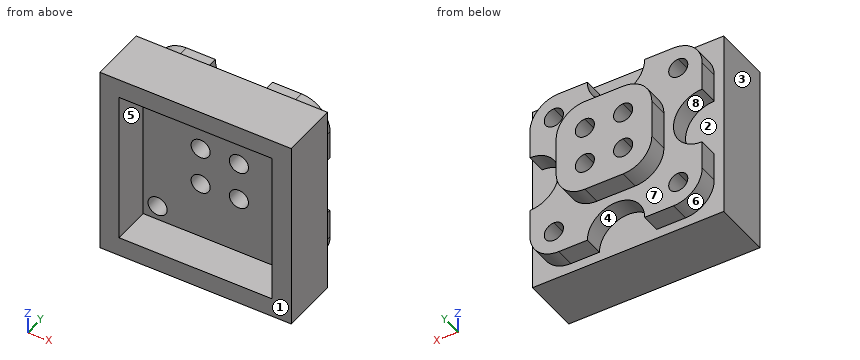
```python
from build123d import *

# Parameters (mm, degrees)
BASE_SQUARE_SKETCH_W        = 100
BASE_SQUARE_SKETCH_H        = 100
BASE_BLOCK_100X100X30_DEPTH = 30
BASE_SHELL_10MM_T           = -10
CROSS_PLATE_SKETCH_R        = 5
CROSS_PLATE_10MM_DEPTH      = 10
PLATE_HOLES_SKETCH_R        = 5
PLATE_ARM_HOLES_4X_DEPTH    = 82.240384046
CENTRE_BOSS_SKETCH_R        = 5
CENTRE_BOSS_10MM_DEPTH      = 10
CENTRE_HOLES_SKETCH_R       = 5
CENTRE_BOSS_HOLES_4X_DEPTH  = 87.602540378


with BuildPart() as part:
    # Base Square Sketch → Base Block 100x100x30 (new body)
    with BuildSketch(Plane(origin=(0, 0, 0), x_dir=(1, 0, 0), z_dir=(0, 1, 0))):
        Rectangle(BASE_SQUARE_SKETCH_W, BASE_SQUARE_SKETCH_H)
    extrude(amount=BASE_BLOCK_100X100X30_DEPTH)

    # Base Shell 10mm
    base_shell_10mm_openings = [part.faces().sort_by_distance(p)[0] for p in [
        (0, 0, 0),
    ]]
    offset(amount=BASE_SHELL_10MM_T, openings=base_shell_10mm_openings, kind=Kind.INTERSECTION)

    # Cross Plate Sketch → Cross Plate 10mm (add)
    with BuildSketch(Plane(origin=(0, 30, 0), x_dir=(1, 0, 0), z_dir=(0, 1, 0))):
        with BuildLine():
            Line((15, 45), (30, 45))
            ThreePointArc((30, 45), (40.606601718, 40.606601718), (45, 30))
            Line((45, 30), (45, 15))
            ThreePointArc((45, 15), (30, 0), (45, -15))
            Line((45, -15), (45, -30))
            ThreePointArc((45, -30), (40.606601718, -40.606601718), (30, -45))
            Line((30, -45), (15, -45))
            ThreePointArc((15, -45), (0, -30), (-15, -45))
            Line((-15, -45), (-30, -45))
            ThreePointArc((-30, -45), (-40.606601718, -40.606601718), (-45, -30))
            Line((-45, -30), (-45, -15))
            ThreePointArc((-45, -15), (-30, 0), (-45, 15))
            Line((-45, 15), (-45, 30))
            ThreePointArc((-45, 30), (-40.606601718, 40.606601718), (-30, 45))
            Line((-30, 45), (-15, 45))
            ThreePointArc((-15, 45), (0, 30), (15, 45))
        make_face()
        with Locations(Location((-32.5, 32.5, 0), (0, 0, 270))):
            Circle(CROSS_PLATE_SKETCH_R, mode=Mode.SUBTRACT)
        with Locations(Location((32.5, 32.5, 0), (0, 0, 270))):
            Circle(CROSS_PLATE_SKETCH_R, mode=Mode.SUBTRACT)
        with Locations(Location((-32.5, -32.5, 0), (0, 0, 270))):
            Circle(CROSS_PLATE_SKETCH_R, mode=Mode.SUBTRACT)
        with Locations(Location((32.5, -32.5, 0), (0, 0, 270))):
            Circle(CROSS_PLATE_SKETCH_R, mode=Mode.SUBTRACT)
    extrude(amount=CROSS_PLATE_10MM_DEPTH)

    # Plate Holes Sketch → Plate Arm Holes 4x (cut, through all)
    with BuildSketch(Plane(origin=(0, 40, 0), x_dir=(1, 0, 0), z_dir=(0, 1, 0))):
        with Locations(Location((-32.5, 32.5, 0), (0, 0, 90))):
            Circle(PLATE_HOLES_SKETCH_R)
        with Locations(Location((32.5, 32.5, 0), (0, 0, 90))):
            Circle(PLATE_HOLES_SKETCH_R)
        with Locations(Location((32.5, -32.5, 0), (0, 0, 90))):
            Circle(PLATE_HOLES_SKETCH_R)
        with Locations(Location((-32.5, -32.5, 0), (0, 0, 90))):
            Circle(PLATE_HOLES_SKETCH_R)
    extrude(amount=-PLATE_ARM_HOLES_4X_DEPTH, mode=Mode.SUBTRACT)

    # Centre Boss Sketch → Centre Boss 10mm (add)
    with BuildSketch(Plane(origin=(0, 40, 0), x_dir=(1, 0, 0), z_dir=(0, 1, 0))):
        with BuildLine():
            Line((-25, 10), (-25, -10))
            ThreePointArc((-25, -10), (-20.606601718, -20.606601718), (-10, -25))
            Line((-10, -25), (10, -25))
            ThreePointArc((10, -25), (20.606601718, -20.606601718), (25, -10))
            Line((25, -10), (25, 10))
            ThreePointArc((25, 10), (20.606601718, 20.606601718), (10, 25))
            Line((10, 25), (-10, 25))
            ThreePointArc((-10, 25), (-20.606601718, 20.606601718), (-25, 10))
        make_face()
        with Locations(Location((-10, 10, 0), (0, 0, 270))):
            Circle(CENTRE_BOSS_SKETCH_R, mode=Mode.SUBTRACT)
        with Locations(Location((10, 10, 0), (0, 0, 270))):
            Circle(CENTRE_BOSS_SKETCH_R, mode=Mode.SUBTRACT)
        with Locations(Location((10, -10, 0), (0, 0, 270))):
            Circle(CENTRE_BOSS_SKETCH_R, mode=Mode.SUBTRACT)
        with Locations(Location((-10, -10, 0), (0, 0, 270))):
            Circle(CENTRE_BOSS_SKETCH_R, mode=Mode.SUBTRACT)
    extrude(amount=CENTRE_BOSS_10MM_DEPTH)

    # Centre Holes Sketch → Centre Boss Holes 4x (cut, through all)
    with BuildSketch(Plane(origin=(0, 50, 0), x_dir=(1, 0, 0), z_dir=(0, 1, 0))):
        with Locations(Location((-10, 10, 0), (0, 0, 90))):
            Circle(CENTRE_HOLES_SKETCH_R)
        with Locations(Location((10, 10, 0), (0, 0, 90))):
            Circle(CENTRE_HOLES_SKETCH_R)
        with Locations(Location((10, -10, 0), (0, 0, 90))):
            Circle(CENTRE_HOLES_SKETCH_R)
        with Locations(Location((-10, -10, 0), (0, 0, 90))):
            Circle(CENTRE_HOLES_SKETCH_R)
    extrude(amount=-CENTRE_BOSS_HOLES_4X_DEPTH, mode=Mode.SUBTRACT)


solid = part.part
```
For this review, take the finished solid that the model builds, in its own axes (mm). Face numbers are marked on the shaded views. A direction names the side the tool comes from. Round coordinates to 2 decimals unless told otherwise and drop trailing zeros. Write each loop counter-clockwise with the first axis right and the second up, starting at its lowest first coordinate (ties: lowest second). Pieces come first, ordered by that corner, then holes. Notation, with made-up numbers: M -9,-1.75 L 5,-1.75 A34 cw 5,34.25 Z; hole C 38,6 d2. An arc over 180 degrees is marked long. One line per item, written item: value. Start each with the question number.
(1) We need section B-B (y = 9.5). Give the boundary of the cut face in (x, z).
(2) We need section A-A (y = 31.5). Count the separate pieces of the cut face and the enclosed holes in it, and give its area (3 significant figures).
(3) The part is to be moulded in two halves that separate along X. For the marked faces 1, 2, 3 and 4, say which applies: released by +X, released by -X, zero draft, split by the parting line, or undercut.
(4) We need section D-D (z = -7.5). Give the boundary of the cut face in (x, y), and give its area (3 significant figures).
(5) Insertion check: pin 1 (6 mm diameter, centred on x = -4.5, y = 36.5, fed in from +Z); pin 2 (8 mm diameter, centred on x = -2, y = 43, fed in from -Z); pin 3 (3 mm diameter, centred on x = -35, z = -12.5, fed in from +Y). Each pin has a flat end and moves straight along its axis. Give the tip position at first contact, or say it passes through.
(6) Machinability: for the marked faces 5, 6, 7 and 8, which of the approach directions +Z, -Z, +X, -X, +Y, -Y give a long, thin tool a straight path to every point of the face, cutting with its end or side? Answer none if there is none.
(7) We need section C-C (x = 0). Give the boundary of the cut face in (y, z), and give its area (3 significant figures).
(8) Wall thickness on line 1 (X direction, y = 23.5, z = -32.5); line 2 (Z direction, x = -32, y = 26); line 3 (Z direction, x = 37, y = 25.5): over which ranges is each line inside the solid? List them lowest first.
Result:
1. outline: M -50,-50 L 50,-50 L 50,50 L -50,50 Z; hole M -40,-40 L 40,-40 L 40,40 L -40,40 Z
2. separate pieces: 1
2. enclosed holes: 8
2. area: 5,860 mm²
3. face 1: zero draft
3. face 2: undercut
3. face 3: released by -X
3. face 4: undercut
4. outline: M -50,0 L -40,0 L -40,20 L -14.33,20 L -14.33,50 L -25,50 L -25,40 L -32.01,40 L -32.01,30 L -50,30 Z; M -5.67,20 L 5.67,20 L 5.67,50 L -5.67,50 Z; M 14.33,20 L 40,20 L 40,0 L 50,0 L 50,30 L 32.01,30 L 32.01,40 L 25,40 L 25,50 L 14.33,50 Z
4. area: 2,020 mm²
5. pin 1: z = 32.01
5. pin 2: z = -30.74
5. pin 3: y = 40
6. face 5: -Y
6. face 6: -Z, -X, +Y
6. face 7: +Y
6. face 8: -X, +Y
7. outline: M 0,-50 L 30,-50 L 30,-30 L 40,-30 L 40,-25 L 50,-25 L 50,25 L 40,25 L 40,30 L 30,30 L 30,50 L 0,50 L 0,40 L 20,40 L 20,-40 L 0,-40 Z
7. area: 2,500 mm²
8. line 1: -50 to -37.5, -27.5 to 27.5, 37.5 to 50
8. line 2: -50 to -37.47, -27.53 to 27.53, 37.47 to 50
8. line 3: -50 to -34.68, -30.32 to 30.32, 34.68 to 50
